```python
from build123d import *

# Parameters (mm, degrees)
SKETCH1_R           = 29
BOSS_EXTRUDE1_DEPTH = 550
CUT_EXTRUDE1_START  = -25
SKETCH2_R           = 29
SKETCH2_R_2         = 24
CUT_EXTRUDE1_DEPTH  = 25
SKETCH3_R           = 20
CUT_EXTRUDE2_DEPTH  = 552.526971235
CHAMFER1_SIZE       = 1
SKETCH4_R           = 24
SKETCH4_R_2         = 22.9
CUT_EXTRUDE3_DEPTH  = 3
FILLET1_R           = 1


with BuildPart() as part:
    # Sketch1 → Boss-Extrude1 (new body)
    with BuildSketch(Plane.XY):
        Circle(SKETCH1_R)
    extrude(amount=BOSS_EXTRUDE1_DEPTH)

    # Sketch2 → Cut-Extrude1 (cut)
    with BuildSketch(Plane.XY.offset(550).offset(CUT_EXTRUDE1_START)):
        Circle(SKETCH2_R)
        Circle(SKETCH2_R_2, mode=Mode.SUBTRACT)
    extrude(amount=CUT_EXTRUDE1_DEPTH, mode=Mode.SUBTRACT)

    # Sketch3 → Cut-Extrude2 (cut, through all)
    with BuildSketch(Plane.XY.offset(550)):
        Circle(SKETCH3_R)
    extrude(amount=-CUT_EXTRUDE2_DEPTH, mode=Mode.SUBTRACT)

    # Chamfer1
    chamfer1_edges = [part.edges().sort_by_distance(p)[0] for p in [
        (-24, 0, 550),
    ]]
    chamfer(chamfer1_edges, length=CHAMFER1_SIZE)

    # Sketch4 → Cut-Extrude3 (cut)
    with BuildSketch(Plane.XY.offset(525)):
        Circle(SKETCH4_R)
        Circle(SKETCH4_R_2, mode=Mode.SUBTRACT)
    extrude(amount=CUT_EXTRUDE3_DEPTH, mode=Mode.SUBTRACT)

    # Fillet1
    fillet1_edges = [part.edges().sort_by_distance(p)[0] for p in [
        (-22.9, 0, 525),
        (-22.9, 0, 528),
    ]]
    fillet(fillet1_edges, radius=FILLET1_R)


solid = part.part
```
The model under review builds one solid part; all positions refer to its coordinate system, in mm. A direction names the side the tool comes from. Round coordinates to 2 decimals unless told otherwise and drop trailing zeros. Loops run counter-clockwise (first coordinate to the right, second up) from the corner with the lowest first, then second, coordinate; pieces in that order, holes last. Notation, with made-up numbers: (83.5, -34.5) - (105.5, -34.5) arc R13 ccw to (105.5, -30.5) - close; hole circle Ø4 at (63, 14.5). An arc over 180 degrees is marked (long way). Write each question's results on one line, items separated by ' | '. Start each with the question number.
Q1. Take a section at C-C on z = 448. Give the boundary of the cut face in (x, y).
Q2. Insertion check: P1, Ø1.5, axis at x = -16.5, z = 329, coming from the +Y side; P2, Ø10, axis at y = -10.5, z = 304, coming from the -X side; P3, Ø6, axis at x = -9, z = 312.5, coming from the +Y side. Each pin has a flat end and moves straight along its axis. Give the tip position at first contact, or say it passes through.
Q3. Take a section at A-A on y = 0. Give the boundary of the cut face in (x, z), plus the area to 3 significant figures.
Q4. Tool access review of faces 1 (the cylindrical face through (-4.964, -22.355, 526.493)), 2 (the cylindrical face through (13.38, -25.73, 258.82)): name each direction out of +Z, -Z, +X, -X, +Y, -Y from which nothing blocks a thin tool from reaching the whole face with its end or side.
Q5. Draft analysis for pull direction Y (two halves, no side actions). For faces 3 (the cylindrical face through (-23.977, 1.055, 538.353)), 4 (the flat face through (-7, -19, 0)), 5 (the cylindrical face through (-4.336, -19.524, 278.85)), state which applies: pulls with the +Y half, pulls with the -Y half, needs draft (parallel to the pull), parting line crosses it, or undercut.
Q6. Wall thickness on line 1 along Y through (x, z) = (0, 158); line 2 along Y through (x, z) = (-2, 346); line 3 along Z through (x, y) = (-20, 15.5): over which ranges is each line inside the solid? List them lowest first. Write a range as [from, to].
Data:
1) outline: circle Ø58 at (0, 0); hole circle Ø40 at (0, 0)
2) P1: stops at y = 24.35 | P2: stops at x = -28.47 | P3: stops at y = 28.37
3) outline: (-29, 0) - (-20, 0) - (-20, 550) - (-23, 550) - (-24, 549) - (-24, 528) - (-23.9, 528) arc R1 cw to (-22.9, 527) - (-22.9, 526) arc R1 cw to (-23.9, 525) - (-29, 525) - close; (20, 0) - (29, 0) - (29, 525) - (23.9, 525) arc R1 cw to (22.9, 526) - (22.9, 527) arc R1 cw to (23.9, 528) - (24, 528) - (24, 549) - (23, 550) - (20, 550) - close | area: 9,640 mm²
4) face 1: none | face 2: +Z, -Z
5) face 3: parting line crosses it | face 4: needs draft | face 5: undercut
6) line 1: y = [-29, -20], [20, 29] | line 2: y = [-28.93, -19.9], [19.9, 28.93] | line 3: z = [0, 525]
